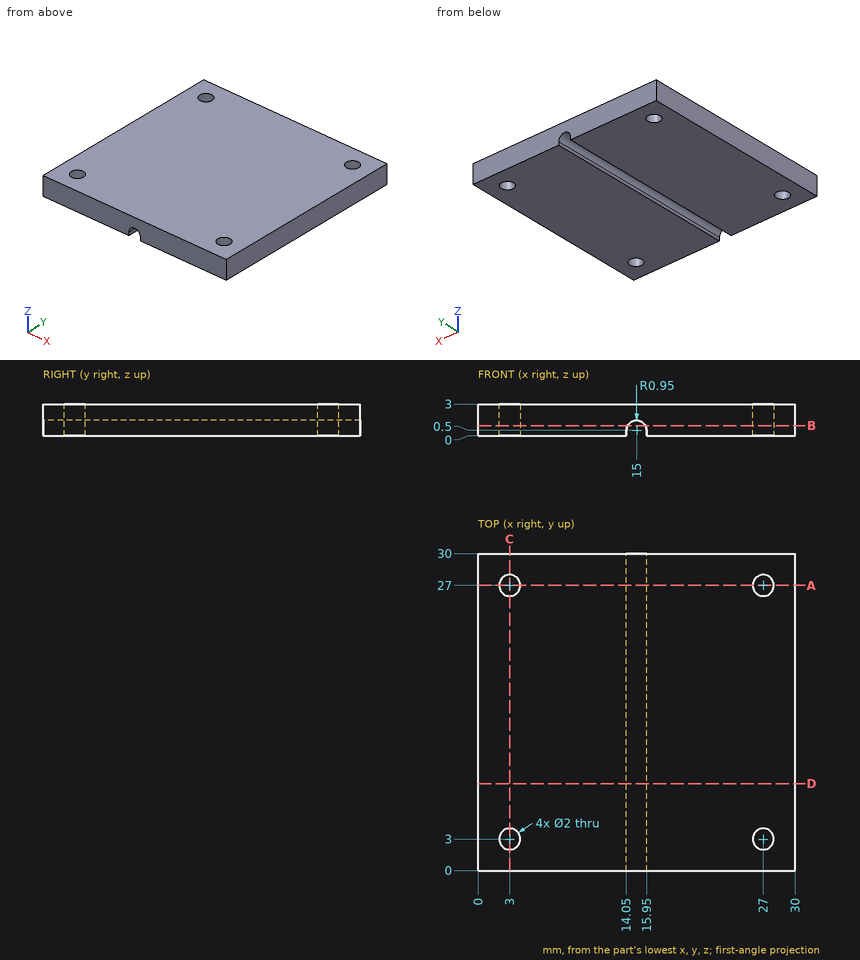
Source: three-view drawing plus pictorial views. Frame: mm from the lowest corner of the part. Coordinates: 2 decimals unless noted, no trailing zeros. Order: outer loops, then holes, each group sorted by start corner. A loop starts at its lowest first (then second) coordinate and runs counter-clockwise, first axis right, second up.
Item 1: Cut plane B-B (z = 0.95). Return loops of the section in (x, y).
Output values:
outline: (0, 0) - (14.16, 0) - (14.16, 30) - (0, 30) - close; (15.84, 0) - (30, 0) - (30, 30) - (15.84, 30) - close; hole circle Ø2 at (3, 3); hole circle Ø2 at (3, 27); hole circle Ø2 at (27, 3); hole circle Ø2 at (27, 27)
Item 2: Material intervals for line 1 (Y direction, x = 27, z = 0.3); line 2 (Y direction, x = 27.75, z = 0.55); line 3 (X direction, y = 6.75, z = 1.15), sorted ascending.
Output values:
line 1: y = 0 to 2, 4 to 26, 28 to 30
line 2: y = 0 to 2.34, 3.66 to 26.34, 27.66 to 30
line 3: x = 0 to 14.31, 15.69 to 30
Item 3: Cut plane A-A (y = 27). Return loops of the section in (x, z).
Output values:
outline: (0, 0) - (2, 0) - (2, 3) - (0, 3) - close; (4, 0) - (14.05, 0) - (14.05, 0.5) arc R0.95 cw to (15.95, 0.5) - (15.95, 0) - (26, 0) - (26, 3) - (4, 3) - close; (28, 0) - (30, 0) - (30, 3) - (28, 3) - close
Item 4: Cut plane C-C (x = 3). Return loops of the section in (y, z).
Output values:
outline: (0, 0) - (2, 0) - (2, 3) - (0, 3) - close; (4, 0) - (26, 0) - (26, 3) - (4, 3) - close; (28, 0) - (30, 0) - (30, 3) - (28, 3) - close
Item 5: Cut plane D-D (y = 8.25). Return loops of the section in (x, z).
Output values:
outline: (0, 0) - (14.05, 0) - (14.05, 0.5) arc R0.95 cw to (15.95, 0.5) - (15.95, 0) - (30, 0) - (30, 3) - (0, 3) - close
